Here's how the part is built. I have some questions about the finished solid (model axes, mm). A direction names the side the tool comes from. Round coordinates to 2 decimals unless told otherwise and drop trailing zeros. Answer in a Markdown table with one row per item.
from build123d import *

# Parameters (mm, degrees)
SKETCH_1_W                     = 800
SKETCH_1_H                     = 80
EXTRUDE_1_DEPTH                = 12
SKETCH_13_W                    = 10
SKETCH_13_H                    = 40
EXTRUDE_2_DEPTH                = 800
CUT_EXTRUDE_1_DEPTH            = 409.881400898
CUT_EXTRUDE_1_DEPTH_BACK       = 409.881400898
SKETCH_15_W                    = 47
SKETCH_15_H                    = 70
CUT_EXTRUDE_2_DEPTH            = 403.968981437
CUT_EXTRUDE_3_DEPTH            = 665.795457265
CUT_EXTRUDE_3_DEPTH_BACK       = 665.795457265
CUT_EXTRUDE_4_DEPTH            = 665.795457265
CUT_EXTRUDE_4_DEPTH_BACK       = 665.795457265
PATTERN_LINEAR_1_COUNT         = 7
PATTERN_LINEAR_1_PITCH         = 82
HOLE_WIZARD_M6_1_2_D           = 6.6
HOLE_WIZARD_M6_1_2_CBORE_D     = 11
HOLE_WIZARD_M6_1_2_CBORE_DEPTH = 6.4
HOLE_WIZARD_5_0_5_1_D          = 5
HOLE_WIZARD_5_0_5_1_DEPTH      = 10
HOLE_WIZARD_5_0_5_1_TIP        = 1.443375673
CUT_EXTRUDE_5_DEPTH            = 10
SKETCH_26_W                    = 663
SKETCH_26_H                    = 18.5
EXTRUDE_3_DEPTH                = 12
CHAMFER_1_SIZE                 = 3
HOLE_WIZARD_M6_2_AT_2_COUNT    = 2
HOLE_WIZARD_M6_2_AT_2_PITCH    = 46
PATTERN_LINEAR_2_COUNT         = 6
PATTERN_LINEAR_2_PITCH         = 100
HOLE_WIZARD_M5_1_D             = 4.2
HOLE_WIZARD_M5_1_DEPTH         = 12.4
HOLE_WIZARD_M5_1_TIP           = 1.2618073
CUT_EXTRUDE_6_DEPTH            = 410.421842126
CUT_EXTRUDE_6_DEPTH_BACK       = 410.421842126
CHAMFER_2_SIZE                 = 1


with BuildPart() as part:
    # 草图1 → 凸台-拉伸1 (new body)
    with BuildSketch(Plane(origin=(0, 0, 0), x_dir=(1, 0, 0), z_dir=(0, 1, 0))):
        Rectangle(SKETCH_1_W, SKETCH_1_H)
    extrude(amount=EXTRUDE_1_DEPTH)

    # 草图13 → 凸台-拉伸2 (add)
    with BuildSketch(Plane(origin=(400, 0, 0), x_dir=(0, 0, -1), z_dir=(1, 0, 0))):
        with Locations((35, -8)):
            Rectangle(SKETCH_13_W, SKETCH_13_H)
    extrude(amount=-EXTRUDE_2_DEPTH)

    # 草图14 → 切除-拉伸1 (cut, two sides: drawn at the far end of the back side and taken through both)
    with BuildSketch(Plane.XY.offset(40).offset(-CUT_EXTRUDE_1_DEPTH_BACK)):
        Polygon((310, 1445.673153531), (310, 12), (310, -39.100998243), (310, -1472.774151774), (3177.346307063, -1472.774151774), (3177.346307063, 1445.673153531), align=None)
    extrude(amount=CUT_EXTRUDE_1_DEPTH + CUT_EXTRUDE_1_DEPTH_BACK, mode=Mode.SUBTRACT)

    # 草图15 → 切除-拉伸2 (cut, through all)
    with BuildSketch(Plane.XZ):
        with Locations((286.5, 5)):
            Rectangle(SKETCH_15_W, SKETCH_15_H)
    extrude(amount=-CUT_EXTRUDE_2_DEPTH, mode=Mode.SUBTRACT)

    # 草图16 → 切除-拉伸3 (cut, two sides: drawn at the far end of the back side and taken through both)
    with BuildSketch(Plane(origin=(263, 0, 0), x_dir=(0, 0, -1), z_dir=(1, 0, 0)).offset(-CUT_EXTRUDE_3_DEPTH_BACK)):
        Polygon((-37.99997, 201.49334526), (-37.99997, 14.161837787), (-37.99997, -5.873299283), (-37.99997, -193.204806756), (-412.662984945, -193.204806756), (-412.662984945, 201.49334526), align=None)
    extrude(amount=CUT_EXTRUDE_3_DEPTH + CUT_EXTRUDE_3_DEPTH_BACK, mode=Mode.SUBTRACT)

    # 草图17 → 切除-拉伸4 (cut, two sides: drawn at the far end of the back side and taken through both)
    with BuildSketch(Plane(origin=(263, 0, 0), x_dir=(0, 0, -1), z_dir=(1, 0, 0)).offset(-CUT_EXTRUDE_4_DEPTH_BACK)):
        Polygon((30, 179.784611671), (30, 12), (30, -28), (30, -195.784611671), (365.569223341, -195.784611671), (365.569223341, 179.784611671), align=None)
    extrude(amount=CUT_EXTRUDE_4_DEPTH + CUT_EXTRUDE_4_DEPTH_BACK, mode=Mode.SUBTRACT)

    # 草图18 → Hole Wizard M6 _1 (revolve, cut)
    with BuildSketch(Plane(origin=(213, 6, -30), x_dir=(0, 1, 0), z_dir=(1, 0, 0))):
        Polygon((0, 0), (0, 15.502151548), (2.5, 14), (2.5, 0), align=None)
    hole_wizard_m6_1 = revolve(axis=Axis((213, 6, -36.35), (0, 0, 1)), mode=Mode.SUBTRACT)

    # 阵列(线性)1: Hole Wizard M6 _1 ×7
    with Locations(*[(-i * PATTERN_LINEAR_1_PITCH, 0, 0) for i in range(1, PATTERN_LINEAR_1_COUNT)]):
        add(hole_wizard_m6_1, mode=Mode.SUBTRACT)

    # Hole Wizard M6 _1 2 (through all)
    with Locations(Plane(origin=(0, 12, 0), x_dir=(1, 0, 0), z_dir=(0, 1, 0))):
        with Locations((-304, 10), (-304, -28)):
            CounterBoreHole(HOLE_WIZARD_M6_1_2_D / 2, HOLE_WIZARD_M6_1_2_CBORE_D / 2, HOLE_WIZARD_M6_1_2_CBORE_DEPTH)

    # Ø5.0 (5) 直径孔1
    with Locations(Plane(origin=(0, 0, -30), x_dir=(-1, 0, 0), z_dir=(0, 0, -1))):
        with Locations((360, 6)):
            Hole(HOLE_WIZARD_5_0_5_1_D / 2, depth=HOLE_WIZARD_5_0_5_1_DEPTH)
            with Locations((0, 0, -(HOLE_WIZARD_5_0_5_1_DEPTH + HOLE_WIZARD_5_0_5_1_TIP / 2))):  # 120° drill point
                Cone(0, HOLE_WIZARD_5_0_5_1_D / 2, HOLE_WIZARD_5_0_5_1_TIP, mode=Mode.SUBTRACT)

    # 草图24 → 切除-拉伸5 (cut)
    with BuildSketch(Plane(origin=(0, 0, -30), x_dir=(-1, 0, 0), z_dir=(0, 0, -1))):
        with BuildLine():
            Line((-227, 3.5), (-233, 3.5))
            ThreePointArc((-233, 3.5), (-235.5, 6), (-233, 8.5))
            Line((-233, 8.5), (-227, 8.5))
            ThreePointArc((-227, 8.5), (-224.5, 6), (-227, 3.5))
        make_face()
    extrude(amount=-CUT_EXTRUDE_5_DEPTH, mode=Mode.SUBTRACT)

    # 草图26 → 凸台-拉伸3 (add)
    with BuildSketch(Plane.XZ):
        with Locations((-68.5, 47.24997)):
            Rectangle(SKETCH_26_W, SKETCH_26_H)
    extrude(amount=-EXTRUDE_3_DEPTH)

    # 倒角1
    chamfer_1_edges = [part.edges().sort_by_distance(p)[0] for p in [
        (-68.5, 0, 56.49997),
    ]]
    chamfer(chamfer_1_edges, length=CHAMFER_1_SIZE)

    # 草图27 → M6 螺纹孔2 (revolve, cut)
    with BuildSketch(Plane(origin=(213, 12, -10), x_dir=(0, 0, 1), z_dir=(1, 0, 0))):
        Polygon((0, 0), (0, 16.502151548), (2.5, 15), (2.5, 0), align=None)
    hole_wizard_m6_2 = revolve(axis=Axis((213, 18.35, -10), (0, -1, 0)), mode=Mode.SUBTRACT)

    # M6 螺纹孔2 at 2: M6 螺纹孔2 ×2
    with Locations(*[(0, 0, i * HOLE_WIZARD_M6_2_AT_2_PITCH) for i in range(1, HOLE_WIZARD_M6_2_AT_2_COUNT)]):
        add(hole_wizard_m6_2, mode=Mode.SUBTRACT)

    # 阵列(线性)2: M6 螺纹孔2 ×6
    with Locations(*[(-i * PATTERN_LINEAR_2_PITCH, 0, 0) for i in range(1, PATTERN_LINEAR_2_COUNT)]):
        add(hole_wizard_m6_2, mode=Mode.SUBTRACT)

    # 阵列(线性)2 copy 1 sketch → 阵列(线性)2 copy 1 (revolve, cut)
    with BuildSketch(Plane(origin=(113, 12, 36), x_dir=(0, 0, 1), z_dir=(1, 0, 0))):
        Polygon((0, 0), (0, 16.502151548), (2.5, 15), (2.5, 0), align=None)
    revolve(axis=Axis((113, 18.35, 36), (0, -1, 0)), mode=Mode.SUBTRACT)

    # 阵列(线性)2 copy 2 sketch → 阵列(线性)2 copy 2 (revolve, cut)
    with BuildSketch(Plane(origin=(13, 12, 36), x_dir=(0, 0, 1), z_dir=(1, 0, 0))):
        Polygon((0, 0), (0, 16.502151548), (2.5, 15), (2.5, 0), align=None)
    revolve(axis=Axis((13, 18.35, 36), (0, -1, 0)), mode=Mode.SUBTRACT)

    # 阵列(线性)2 copy 3 sketch → 阵列(线性)2 copy 3 (revolve, cut)
    with BuildSketch(Plane(origin=(-87, 12, 36), x_dir=(0, 0, 1), z_dir=(1, 0, 0))):
        Polygon((0, 0), (0, 16.502151548), (2.5, 15), (2.5, 0), align=None)
    revolve(axis=Axis((-87, 18.35, 36), (0, -1, 0)), mode=Mode.SUBTRACT)

    # 阵列(线性)2 copy 4 sketch → 阵列(线性)2 copy 4 (revolve, cut)
    with BuildSketch(Plane(origin=(-187, 12, 36), x_dir=(0, 0, 1), z_dir=(1, 0, 0))):
        Polygon((0, 0), (0, 16.502151548), (2.5, 15), (2.5, 0), align=None)
    revolve(axis=Axis((-187, 18.35, 36), (0, -1, 0)), mode=Mode.SUBTRACT)

    # 阵列(线性)2 copy 5 sketch → 阵列(线性)2 copy 5 (revolve, cut)
    with BuildSketch(Plane(origin=(-287, 12, 36), x_dir=(0, 0, 1), z_dir=(1, 0, 0))):
        Polygon((0, 0), (0, 16.502151548), (2.5, 15), (2.5, 0), align=None)
    revolve(axis=Axis((-287, 18.35, 36), (0, -1, 0)), mode=Mode.SUBTRACT)

    # M5 螺纹孔1
    with Locations(Plane.XY.offset(56.49997)):
        with Locations((-312.000000001, 6.5), (-292.000000001, 6.5), (-272.000000001, 6.5)):
            Hole(HOLE_WIZARD_M5_1_D / 2, depth=HOLE_WIZARD_M5_1_DEPTH)
            with Locations((0, 0, -(HOLE_WIZARD_M5_1_DEPTH + HOLE_WIZARD_M5_1_TIP / 2))):  # 118° drill point
                Cone(0, HOLE_WIZARD_M5_1_D / 2, HOLE_WIZARD_M5_1_TIP, mode=Mode.SUBTRACT)

    # 草图31 → 切除-拉伸6 (cut, two sides: drawn at the far end of the back side and taken through both)
    with BuildSketch(Plane.XY.offset(56.49997).offset(-CUT_EXTRUDE_6_DEPTH_BACK)):
        Polygon((-370, 1306.901366583), (-370, 26.75), (-370, -39.304225055), (-370, -1319.455591638), (-2930.302733167, -1319.455591638), (-2930.302733167, 1306.901366583), align=None)
    extrude(amount=CUT_EXTRUDE_6_DEPTH + CUT_EXTRUDE_6_DEPTH_BACK, mode=Mode.SUBTRACT)

    # 倒角2
    chamfer_2_edges = [part.edges().sort_by_distance(p)[0] for p in [
        (263, 7.5, 56.49997),
        (-370, 6, -30),
        (-370, 7.5, 56.49997),
        (263, 6, -30),
    ]]
    chamfer(chamfer_2_edges, length=CHAMFER_2_SIZE)


solid = part.part
1) Which directions (+Z, -Z, +X, -X, +Y, -Y) give clear straight access to the entire face, cutting with the end or side of a thin tool? Please do faces 4 (the face through (-298.754, 8.845, 26.348)), 5 (the face through (263, 6, 13)).
Response:
| item | result |
|---|---|
| face 4 | +Y |
| face 5 | +Z, -Z, +X, +Y, -Y |
2) For pin 1 (4 mm diameter, centred on x = -360, y = 6, fed in from -Z); pin 2 (6 mm diameter, centred on x = -304, z = 28, fed in from +Y); pin 3 (3.5 mm diameter, centred on x = -312, y = 6.5, fed in from +Z); pin 4 (7.5 mm diameter, centred on x = -304, z = -10, fed in from +Y), each with a flat end and sliding along its axis, tell me the tip position at first contact or that it passes through.
Response:
| item | result |
|---|---|
| pin 1 | stops at z = -19.71 |
| pin 2 | passes through |
| pin 3 | stops at z = 43.89 |
| pin 4 | stops at y = 5.6 |
3) We'd pull the mould along Z, two halves only. Please class faces 1 (the face through (-370, 6, 13)), 2 (the face through (-58, 6, -30)), 3 (the face through (-304, 5.6, -6)): +Z half, -Z half, draft (parallel to the pull), parting line (faces both ways), or undercut.
Response:
| item | result |
|---|---|
| face 1 | draft |
| face 2 | -Z half |
| face 3 | undercut |
4) I need wall thicknesses on line 1 (Z direction, x = -305, y = 7); line 2 (X direction, y = 8, z = 28); line 3 (Z direction, x = -287, y = 4.5). Which ranges of each line are inside material? Lowest first, please. Write a range as [from, to].
Response:
| item | result |
|---|---|
| line 1 | z = [-30, -15.41], [-4.59, 22.59], [33.41, 56.5] |
| line 2 | x = [-370, -309.5], [-298.5, 263] |
| line 3 | z = [-30, -12.5], [-7.5, 33.5], [38.5, 56.5] |
